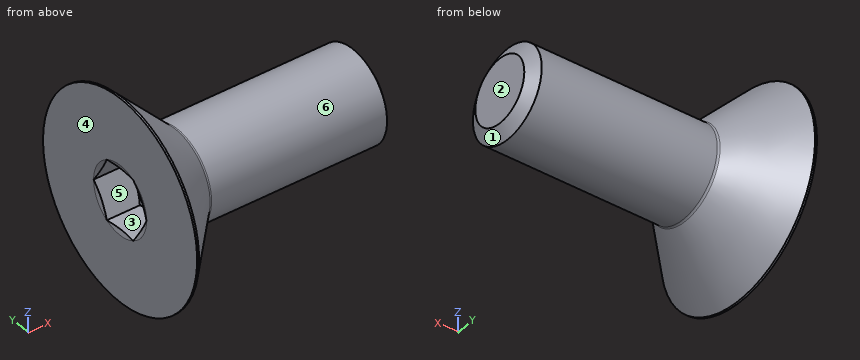
from build123d import *

# Parameters (mm, degrees)
CUT_EXTRUDE1_DEPTH = 1.96


with BuildPart() as part:
    # Sketch1 → Revolve1 (revolve)
    with BuildSketch(Plane.XY):
        with BuildLine():
            Line((0, 1.5), (-6.097552518, 1.5))
            ThreePointArc((-6.097552518, 1.5), (-6.136625631, 1.507949515), (-6.169486498, 1.530534163))
            Line((-6.169486498, 1.530534163), (-7.936181121, 3.36))
            Line((-7.936181121, 3.36), (-8, 3.36))
            Line((-8, 3.36), (-8, 0))
            Line((-8, 0), (0, 0))
            Line((0, 0), (0, 1.5))
        make_face()
    revolve(axis=Axis((0, 0, 0), (-1, 0, 0)))

    # Sketch2 → Cut-Extrude1 (cut)
    with BuildSketch(Plane.ZY.offset(8)):
        Polygon((0, 1.154700538), (-1, 0.577350269), (-1, -0.577350269), (0, -1.154700538), (1, -0.577350269), (1, 0.577350269), align=None)
    extrude(amount=-CUT_EXTRUDE1_DEPTH, mode=Mode.SUBTRACT)

    # Sketch6 → Revolve2 (revolve)
    with BuildSketch(Plane.XY, mode=Mode.PRIVATE) as revolve2_sk:
        Polygon((-6.9, 1.154700538), (-6.233333333, 0), (-5.74, 0), (-5.74, 1.154700538), align=None)
    revolve(revolve2_sk.sketch.rotate(Axis((-8, 0, 0), (1, 0, 0)), 90), axis=Axis((-8, 0, 0), (1, 0, 0)))

    # Sketch7 → Cut-Revolve2 (revolve, cut)
    with BuildSketch(Plane.XY):
        Polygon((-8, 1.154700538), (-8, 0), (-7.67, 0), align=None)
    revolve(axis=Axis((-8, 0, 0), (1, 0, 0)), mode=Mode.SUBTRACT)

    # Sketch4 → Cut-Revolve1 (revolve, cut)
    with BuildSketch(Plane.XY):
        Polygon((-0.25, 1.5), (0, 1.066987298), (0.25, 1.5), align=None)
    revolve(axis=Axis((-0.25, 0, 0), (1, 0, 0)), mode=Mode.SUBTRACT)


solid = part.part
Geometry check sheet. Reference: the model listing, model coordinates, mm. Face numbers are marked on the shaded views. A direction names the side the tool comes from. Round coordinates to 2 decimals unless told otherwise and drop trailing zeros. Loops run counter-clockwise (first coordinate to the right, second up) from the corner with the lowest first, then second, coordinate; pieces in that order, holes last. Notation, with made-up numbers: (51, 80.5) - (91, 80.5) arc R12 ccw to (91, 84.5) - close; hole circle Ø8 at (38, -30.75). An arc over 180 degrees is marked (long way). One line per question, with ' | ' between items. Start each with the question number.
1. Cross-section at B-B on x = -6.5. Record the cut outline in (y, z).
2. Draft check along Y on the marked faces 1, 2 and 3. Enter one of: released by +Y, released by -Y, zero draft, split by the parting line, or undercut.
3. Depth check by flat-ended pin: pin 1 (4 mm diameter, centred on x = -5, z = -0.5, fed in from -Y); pin 2 (1 mm diameter, centred on x = -2, y = -1.5, fed in from +Z); pin 3 (0.6 mm diameter, centred on x = -7.5, y = 0, fed in from -Z). Enter the tip coordinate at first touch or a pass-through.
4. Cross-section at A-A on x = -5.5. Record the cut outline in (y, z).
5. Scan lines: line 1 (Y direction, x = -1.25, z = 0); line 2 (X direction, y = 0, z = -2.5). Record each from-to range of solid material in increasing order. Write a range as [from, to].
6. Tool access check on the marked faces 4, 5 and 6. Record the directions out of +Z, -Z, +X, -X, +Y, -Y that give a thin tool (end or side, any length) a straight path to the whole face; none if there is none.
Taken from the geometry:
1) outline: circle Ø3.75 at (0, 0); hole circle Ø0.92 at (0, 0)
2) face 1: split by the parting line | face 2: zero draft | face 3: undercut
3) pin 1: y = -2.36 | pin 2: z = 1.12 | pin 3: z = -3.22
4) outline: circle Ø3 at (0, 0)
5) line 1: [-1.5, 1.5] | line 2: [-8, -7.11]
6) face 4: +Z, -Z, -X, +Y, -Y | face 5: -X | face 6: +X
